from build123d import *


with BuildPart() as part:
    # Sketch1 → Revolve-Thin1 (revolve)
    with BuildSketch(Plane.XY, mode=Mode.PRIVATE) as revolve_thin1_sk:
        with BuildLine():
            Line((-2.18, 21.493868799), (-2.18, 16.993868799))
            ThreePointArc((-2.18, 16.993868799), (-1.876352845, 15.884048994), (-1.05, 15.083397653))
            Line((-1.05, 15.083397653), (-1.05, 7.910471146))
            ThreePointArc((-1.05, 7.910471146), (-1.876352845, 7.109819805), (-2.18, 6))
            Line((-2.18, 6), (-2.18, 0))
            Line((-2.18, 0), (-2.68, 0))
            Line((-2.68, 0), (-2.68, 6))
            ThreePointArc((-2.68, 6), (-2.380798185, 7.230528342), (-1.55, 8.186298241))
            Line((-1.55, 8.186298241), (-1.55, 14.807570558))
            ThreePointArc((-1.55, 14.807570558), (-2.380798185, 15.763340457), (-2.68, 16.993868799))
            Line((-2.68, 16.993868799), (-2.68, 21.493868799))
            Line((-2.68, 21.493868799), (-2.18, 21.493868799))
        make_face()
    revolve(revolve_thin1_sk.sketch.rotate(Axis((0, 24.17230999, 0), (0, -1, 0)), 270), axis=Axis((0, 24.17230999, 0), (0, -1, 0)))


solid = part.part
For this review, take the finished solid that the model builds, in its own axes (mm). A direction names the side the tool comes from. Round coordinates to 2 decimals unless told otherwise and drop trailing zeros. Order: outer loops, then holes, each group sorted by start corner. A loop starts at its lowest first (then second) coordinate and runs counter-clockwise, first axis right, second up. Notation, with made-up numbers: M 11,13.5 L 40,13.5 A31 ccw 40,41.5 Z; hole C 22,22.5 d8. An arc over 180 degrees is marked long. Use a Markdown table: item, result. Add a question column.
Item 1: To check wall thickness, follow line 1 along X through (y, z) = (4.45, 0); line 2 along X through (y, z) = (8.5, 0.75); line 3 along Y through (x, z) = (1.2, -1.25). State the ranges of each line that lie inside material, in increasing order.
Item 2: Insertion check: pin 1 (1.5 mm diameter, centred on y = 18.5, z = 1, fed in from +X); pin 2 (2 mm diameter, centred on y = 14.5, z = 1, fed in from -X); pin 3 (1 mm diameter, centred on x = -2, z = 0, fed in from -Y); pin 4 (2.5 mm diameter, centred on x = 0, z = 0, fed in from +Y). Each pin has a flat end and moves straight along its axis. Give the tip position at first contact, or say it passes through.
Item 3: Add section C-C, the plane x = 1.3. Give the boundary of the cut face in (y, z).
Item 4: Add section B-B, the plane z = 0. Give the boundary of the cut face in (x, y), then the cut area to 3 significant figures.
Item 5: Tool access review of faces 1 (the cylindrical face through (-0.65, 19.21, 2.08)), 2 (the cylindrical face through (-0.32, 11.45, 1)), 3 (the cylindrical face through (-0.466, 11.543, 1.478)): name each direction out of +Z, -Z, +X, -X, +Y, -Y from which nothing blocks a thin tool from reaching the whole face with its end or side.
Item 6: Add section D-D, the plane y = 15.5. Give the boundary of the cut face in (x, z).
Item 7: Mouldability with a two-part tool opening along Z and no side actions: class faces 4 (the cylindrical face through (-2.657, 19.275, -0.349)), 5 (the cylindrical face through (-0.65, 2.96, 2.08)) as released by +Z, released by -Z, zero draft, split by the parting line, or undercut.
Item 8: Add section A-A, the plane x = 0. Give the boundary of the cut face in (y, z).
Geometry results:
| question | item | result |
|---|---|---|
| 1 | line 1 | x = -2.68 to -2.18, 2.18 to 2.68 |
| 1 | line 2 | x = -1.36 to -0.73, 0.73 to 1.36 |
| 1 | line 3 | y = 7.32 to 8.04, 14.95 to 15.67 |
| 2 | pin 1 | stops at x = 2.67 |
| 2 | pin 2 | stops at x = -2.08 |
| 2 | pin 3 | stops at y = 0 |
| 2 | pin 4 | stops at y = 15.21 |
| 3 | outline | M 0,-2.34 L 6,-2.34 A2.34 ccw 8.19,-0.84 L 14.81,-0.84 A2.34 ccw 16.99,-2.34 L 21.49,-2.34 L 21.49,-1.75 L 16.99,-1.75 A1.75 cw 16.99,1.75 L 21.49,1.75 L 21.49,2.34 L 16.99,2.34 A2.34 ccw 14.81,0.84 L 8.19,0.84 A2.34 ccw 6,2.34 L 0,2.34 L 0,1.75 L 6,1.75 A1.75 cw 6,-1.75 L 0,-1.75 Z |
| 4 | outline | M -2.68,0 L -2.18,0 L -2.18,6 A2.18 cw -1.05,7.91 L -1.05,15.08 A2.18 cw -2.18,16.99 L -2.18,21.49 L -2.68,21.49 L -2.68,16.99 A2.68 ccw -1.55,14.81 L -1.55,8.19 A2.68 ccw -2.68,6 Z; M 1.05,7.91 A2.18 cw 2.18,6 L 2.18,0 L 2.68,0 L 2.68,6 A2.68 ccw 1.55,8.19 L 1.55,14.81 A2.68 ccw 2.68,16.99 L 2.68,21.49 L 2.18,21.49 L 2.18,16.99 A2.18 cw 1.05,15.08 Z |
| 4 | area | 22.3 mm² |
| 5 | face 1 | +Y |
| 5 | face 2 | +Y, -Y |
| 5 | face 3 | none |
| 6 | outline | C 0,0 d4.45; hole C 0,0 d3.18 |
| 7 | face 4 | split by the parting line |
| 7 | face 5 | undercut |
| 8 | outline | M 0,-2.68 L 6,-2.68 A2.68 ccw 8.19,-1.55 L 14.81,-1.55 A2.68 ccw 16.99,-2.68 L 21.49,-2.68 L 21.49,-2.18 L 16.99,-2.18 A2.18 cw 15.08,-1.05 L 7.91,-1.05 A2.18 cw 6,-2.18 L 0,-2.18 Z; M 0,2.18 L 6,2.18 A2.18 cw 7.91,1.05 L 15.08,1.05 A2.18 cw 16.99,2.18 L 21.49,2.18 L 21.49,2.68 L 16.99,2.68 A2.68 ccw 14.81,1.55 L 8.19,1.55 A2.68 ccw 6,2.68 L 0,2.68 Z |
